The model under review builds one solid part; all positions refer to its coordinate system, in mm. A direction names the side the tool comes from. Round coordinates to 2 decimals unless told otherwise and drop trailing zeros. Write each loop counter-clockwise with the first axis right and the second up, starting at its lowest first coordinate (ties: lowest second). Pieces come first, ordered by that corner, then holes.
Item 1: To check wall thickness, follow L1, parallel to Y at x = 75, z = 14; L2, parallel to Y at x = -72.5, z = 1.75; L3, parallel to X at y = 23.5, z = 4.5. State the ranges of each line that lie inside material, in increasing order.
Item 2: Add section C-C (x = -75). Give the boundary of the cut face in (y, z).
Item 3: Add section A-A (y = 60). Give the boundary of the cut face in (x, z).
Item 4: Add section B-B (x = 60). Give the boundary of the cut face in (y, z), plus the area to 3 significant figures.
Item 5: Add section D-D (z = 13.75). State how many separate pieces and enclosed holes the cut face has, plus the area to 3 significant figures.
Item 6: Draft analysis for pull direction Y (two halves, no side actions). For faces 3 (the face through (-1, -67.5, 10)), 4 (the face through (95, -1, 10)), 5 (the face through (65.7, 41.02, 9.86)), state which applies: +Y half, -Y half, draft (parallel to the pull), parting line (faces both ways), or undercut.
Item 7: Machinability: for faces 1 (the face through (-51.23, 28.5, 9.99)), 2 (the face through (-1, 1, 0)), which of the approach directions +Z, -Z, +X, -X, +Y, -Y give a long, thin tool a straight path to every point of the face, cutting with its end or side? Answer none if there is none.
Item 8: Clearance check with a flat-ended pin moving along its axis: pin 1 Ø4.5 at (x, y) = (60, 60) entering from +Z. State where the tip first meets the part, or that it passes through.
```python
from build123d import *

# Parameters (mm, degrees)
SKETCH1_W             = 190
SKETCH1_H             = 135
SKETCH1_R             = 12.611940299
BOSS_EXTRUDE1_DEPTH   = 20
M6_TAPPED_HOLE6_D     = 5
M8_TAPPED_HOLE1_D     = 6.8
M8_TAPPED_HOLE1_DEPTH = 19.75
M8_TAPPED_HOLE1_TIP   = 2.042926105


with BuildPart() as part:
    # Sketch1 → Boss-Extrude1 (new body)
    with BuildSketch(Plane.XY):
        Rectangle(SKETCH1_W, SKETCH1_H)
        with Locations((-75, 32.5)):
            Circle(SKETCH1_R, mode=Mode.SUBTRACT)
        with Locations((-75, -32.5)):
            Circle(SKETCH1_R, mode=Mode.SUBTRACT)
        with Locations((75, 32.5)):
            Circle(SKETCH1_R, mode=Mode.SUBTRACT)
        with Locations((75, -32.5)):
            Circle(SKETCH1_R, mode=Mode.SUBTRACT)
    extrude(amount=BOSS_EXTRUDE1_DEPTH)

    # M6 Tapped Hole6 (through all)
    with Locations(Plane(origin=(0, 0, 0), x_dir=(-1, 0, 0), z_dir=(0, 0, -1))):
        with Locations((-60, 60), (60, 60)):
            Hole(M6_TAPPED_HOLE6_D / 2)

    # M8 Tapped Hole1
    with Locations(Plane.XY.offset(20)):
        with Locations((-51.96743603, 31.820881882), (-51.96743603, -34.622720538), (52.234277806, -34.622720538), (52.234277806, 31.820881882)):
            Hole(M8_TAPPED_HOLE1_D / 2, depth=M8_TAPPED_HOLE1_DEPTH)
            with Locations((0, 0, -(M8_TAPPED_HOLE1_DEPTH + M8_TAPPED_HOLE1_TIP / 2))):  # 118° drill point
                Cone(0, M8_TAPPED_HOLE1_D / 2, M8_TAPPED_HOLE1_TIP, mode=Mode.SUBTRACT)


solid = part.part
```
Numbers:
1. L1: y = -67.5 to -45.11, -19.89 to 19.89, 45.11 to 67.5
1. L2: y = -67.5 to -44.86, -20.14 to 20.14, 44.86 to 67.5
1. L3: x = -95 to -83.84, -66.16 to 66.16, 83.84 to 95
2. outline: (-67.5, 0) - (-45.11, 0) - (-45.11, 20) - (-67.5, 20) - close; (-19.89, 0) - (19.89, 0) - (19.89, 20) - (-19.89, 20) - close; (45.11, 0) - (67.5, 0) - (67.5, 20) - (45.11, 20) - close
3. outline: (-95, 0) - (-62.5, 0) - (-62.5, 20) - (-95, 20) - close; (-57.5, 0) - (57.5, 0) - (57.5, 20) - (-57.5, 20) - close; (62.5, 0) - (95, 0) - (95, 20) - (62.5, 20) - close
4. outline: (-67.5, 0) - (57.5, 0) - (57.5, 20) - (-67.5, 20) - close; (62.5, 0) - (67.5, 0) - (67.5, 20) - (62.5, 20) - close
4. area: 2,600 mm2
5. separate pieces: 1
5. enclosed holes: 10
5. area: 23,500 mm2
6. face 3: -Y half
6. face 4: draft
6. face 5: undercut
7. face 1: +Z
7. face 2: -Z, +X, -X, +Y, -Y
8. pin 1: passes through
